Model file for the job. Use its own axes, mm. Face numbers are marked on the shaded views. Coordinates: 2 decimals unless noted, no trailing zeros. Order: outer loops, then holes, each group sorted by start corner. A loop starts at its lowest first (then second) coordinate and runs counter-clockwise, first axis right, second up.
from build123d import *

# Parameters (mm, degrees)
SKETCH_1_W              = 100
SKETCH_1_H              = 140
EXTRUDE_1_DEPTH         = 20
HOLE_WIZARD_M10_1_D     = 8.5
HOLE_WIZARD_M10_1_DEPTH = 24.5
HOLE_WIZARD_M10_1_TIP   = 2.553657631
SKETCH_4_R              = 20
CUT_EXTRUDE_1_DEPTH     = 12
SKETCH_5_R              = 17.5
CUT_EXTRUDE_2_DEPTH     = 87.856203002
HOLE_WIZARD_M8_1_D      = 6.8
HOLE_WIZARD_M6_1_D      = 5
HOLE_WIZARD_M6_1_DEPTH  = 15
HOLE_WIZARD_M6_1_TIP    = 1.502151548


with BuildPart() as part:
    # 草图1 → 凸台-拉伸1 (new body)
    with BuildSketch(Plane(origin=(0, 0, 0), x_dir=(0, 0, -1), z_dir=(1, 0, 0))):
        Rectangle(SKETCH_1_W, SKETCH_1_H)
    extrude(amount=EXTRUDE_1_DEPTH)

    # M10 螺纹孔1
    with Locations(Plane(origin=(0, -70, 0), x_dir=(-1, 0, 0), z_dir=(0, -1, 0))):
        with Locations((-10, 30), (-10, -30)):
            Hole(HOLE_WIZARD_M10_1_D / 2, depth=HOLE_WIZARD_M10_1_DEPTH)
            with Locations((0, 0, -(HOLE_WIZARD_M10_1_DEPTH + HOLE_WIZARD_M10_1_TIP / 2))):  # 118° drill point
                Cone(0, HOLE_WIZARD_M10_1_D / 2, HOLE_WIZARD_M10_1_TIP, mode=Mode.SUBTRACT)

    # 草图4 → 切除-拉伸1 (cut)
    with BuildSketch(Plane(origin=(20, 0, 0), x_dir=(0, 0, -1), z_dir=(1, 0, 0))):
        with Locations((0, 30)):
            Circle(SKETCH_4_R)
    extrude(amount=-CUT_EXTRUDE_1_DEPTH, mode=Mode.SUBTRACT)

    # 草图5 → 切除-拉伸2 (cut, through all)
    with BuildSketch(Plane(origin=(8, 0, 0), x_dir=(0, 0, -1), z_dir=(1, 0, 0))):
        with Locations((0, 30)):
            Circle(SKETCH_5_R)
    extrude(amount=-CUT_EXTRUDE_2_DEPTH, mode=Mode.SUBTRACT)

    # M8 螺纹孔1 (through all)
    with Locations(Plane.ZY):
        with Locations((-30, 55), (30, 55), (-30, 5), (30, 5)):
            Hole(HOLE_WIZARD_M8_1_D / 2)

    # M6 螺纹孔1
    with Locations(Plane(origin=(0, 70, 0), x_dir=(1, 0, 0), z_dir=(0, 1, 0))):
        with Locations((10, 30), (10, -30)):
            Hole(HOLE_WIZARD_M6_1_D / 2, depth=HOLE_WIZARD_M6_1_DEPTH)
            with Locations((0, 0, -(HOLE_WIZARD_M6_1_DEPTH + HOLE_WIZARD_M6_1_TIP / 2))):  # 118° drill point
                Cone(0, HOLE_WIZARD_M6_1_D / 2, HOLE_WIZARD_M6_1_TIP, mode=Mode.SUBTRACT)


solid = part.part
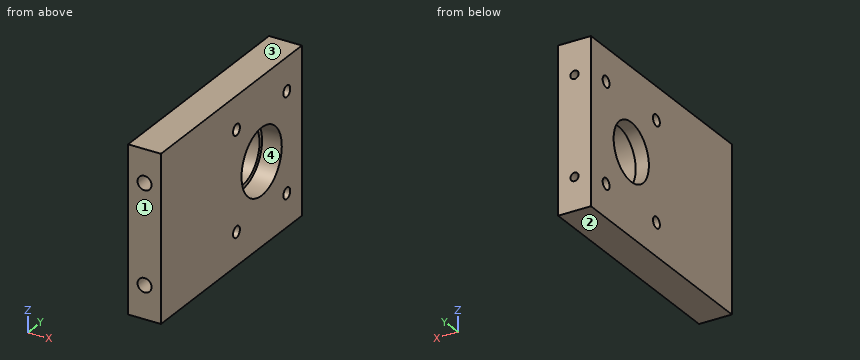
Q1. Cut at B-B, the plane z = 0. List the corners of the cut face in (x, y).
Established:
outline: (0, -70) - (20, -70) - (20, 10) - (8, 10) - (8, 12.5) - (0, 12.5) - close; (0, 47.5) - (8, 47.5) - (8, 50) - (20, 50) - (20, 70) - (0, 70) - close
Q2. Probe line 1 (Z direction, x = 9.5, y = -60); line 2 (Z direction, x = 10, y = 67.5); line 3 (Y direction, x = 5.5, z = 11.5). List the from-to ranges inside material, lowest first.
Established:
line 1: z = -50 to -34.22, -25.78 to 25.78, 34.22 to 50
line 2: z = -50 to -32.5, -27.5 to 27.5, 32.5 to 50
line 3: y = -70 to 16.81, 43.19 to 70
Q3. Mould opens along Z. For the marked faces 1, 2, 3 and 4 say: pulls with the +Z half, pulls with the -Z half, needs draft (parallel to the pull), parting line crosses it, or undercut.
Established:
face 1: needs draft
face 2: pulls with the -Z half
face 3: pulls with the +Z half
face 4: undercut
Q4. Cut at D-D, the plane y = -52. List the corners of the cut face in (x, z).
Established:
outline: (0, -50) - (20, -50) - (20, 50) - (0, 50) - close; hole circle Ø8.5 at (10, -30); hole circle Ø8.5 at (10, 30)
Q5. Drop flat-ended pins along their axis: P1, Ø4, axis at x = 10, z = -30, coming from the +Y side; P2, Ø3, axis at x = 10, z = 30, coming from the -Y side; P3, Ø20, axis at y = 39.5, z = 3.5, coming from the +X side. Give the stop position or say it passes through.
Established:
P1: stops at y = 52.25
P2: stops at y = -43.85
P3: stops at x = 20
Q6. Cut at A-A, the plane y = 55. List the corners of the cut face in (x, z), plus the area to 3 significant figures.
Established:
outline: (0, -50) - (20, -50) - (20, -33.4) - (0, -33.4) - close; (0, -26.6) - (20, -26.6) - (20, 26.6) - (0, 26.6) - close; (0, 33.4) - (20, 33.4) - (20, 50) - (0, 50) - close
area: 1,730 mm2
Q7. Cut at C-C, the plane x = 17.25. List the corners of the cut face in (y, z).
Established:
outline: (-70, -50) - (70, -50) - (70, 50) - (-70, 50) - close; hole circle Ø6.8 at (5, -30); hole circle Ø6.8 at (5, 30); hole circle Ø40 at (30, 0); hole circle Ø6.8 at (55, -30); hole circle Ø6.8 at (55, 30)
